Verification items for the finished model (mm, model axes). Face numbers are marked on the shaded views. Round coordinates to 2 decimals unless told otherwise and drop trailing zeros. Write each loop counter-clockwise with the first axis right and the second up, starting at its lowest first coordinate (ties: lowest second). Pieces come first, ordered by that corner, then holes. Notation, with made-up numbers: (58.25, 66.5) - (83.25, 66.5) arc R23 ccw to (83.25, 85.5) - close; hole circle Ø7 at (23, 75). An arc over 180 degrees is marked (long way). Answer as a JSON object with one key per item and string values.
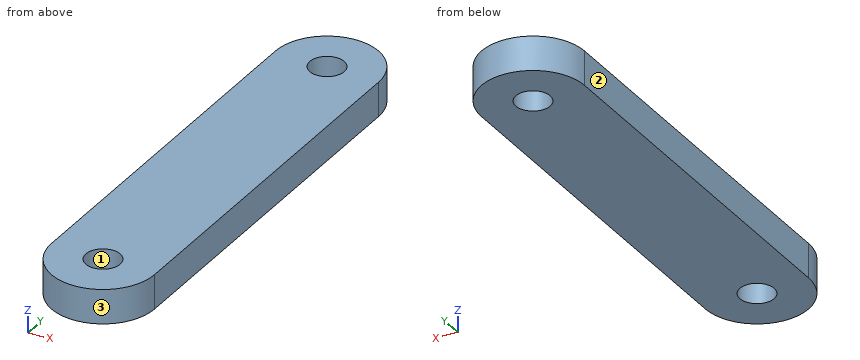
```python
from build123d import *

# Parameters (mm, degrees)
SKETCH_1_R      = 5
EXTRUDE_1_DEPTH = 10


with BuildPart() as part:
    # 草图1 → 凸台-拉伸1 (new body)
    with BuildSketch(Plane.XY):
        with BuildLine():
            Line((-15, 0), (-15, 110))
            ThreePointArc((-15, 110), (0, 125), (15, 110))
            Line((15, 110), (15, 0))
            ThreePointArc((15, 0), (0, -15), (-15, 0))
        make_face()
        Circle(SKETCH_1_R, mode=Mode.SUBTRACT)
        with Locations((0, 110)):
            Circle(SKETCH_1_R, mode=Mode.SUBTRACT)
    extrude(amount=EXTRUDE_1_DEPTH)


solid = part.part
```
1. Cross-section at A-A (x = 0). Record the boundary of the cut face in (y, z).
Completed:
{"outline": "(-15, 0) - (-5, 0) - (-5, 10) - (-15, 10) - close; (5, 0) - (105, 0) - (105, 10) - (5, 10) - close; (115, 0) - (125, 0) - (125, 10) - (115, 10) - close"}
2. Mould release check, pull along Y, two halves, no side actions. Record for the marked faces 1, 2 and 3: released by +Y, released by -Y, zero draft, split by the parting line, or undercut.
Completed:
{"face 1": "undercut", "face 2": "zero draft", "face 3": "released by -Y"}
3. Cross-section at B-B (z = 6.5). Record the boundary of the cut face in (x, y), plus the area to 3 significant figures.
Completed:
{"outline": "(-15, 0) arc R15 ccw to (15, 0) - (15, 110) arc R15 ccw to (-15, 110) - close; hole circle Ø10 at (0, 0); hole circle Ø10 at (0, 110)", "area": "3,850 mm^2"}
4. Cross-section at C-C (x = -12). Record the boundary of the cut face in (y, z), plus the area to 3 significant figures.
Completed:
{"outline": "(-9, 0) - (119, 0) - (119, 10) - (-9, 10) - close", "area": "1,280 mm^2"}
5. Material ranges on probe 1 along Y at (x, z) = (0, 7); probe 2 along Y at (x, z) = (3, 9); probe 3 along X at (y, z) = (114.5, 6.75), recorded low to high. Write a range as from..to.
Completed:
{"probe 1": "y = -15..-5, 5..105, 115..125", "probe 2": "y = -14.7..-4, 4..106, 114..124.7", "probe 3": "x = -14.31..-2.18, 2.18..14.31"}
6. Go/stop test with flat-tipped pins: pin 1 (4 mm diameter, centred on x = 5.5, z = 1.5, fed in from +Y); pin 2 (2 mm diameter, centred on x = 5, z = 2, fed in from -Y); pin 3 (6 mm diameter, centred on x = -9, z = 4, fed in from +Y); pin 4 (9 mm diameter, centred on x = 0, y = 110, fed in from +Z). Record where each tip stops, or that it passes through.
Completed:
{"pin 1": "stops at y = 124.59", "pin 2": "stops at y = -14.46", "pin 3": "stops at y = 123.75", "pin 4": "passes through"}
